Geometry check sheet. Reference: the model listing, model coordinates, mm. Face numbers are marked on the shaded views. A direction names the side the tool comes from. Give positions to 0.01 mm unless a question says otherwise; leave off trailing zeros. Write each loop counter-clockwise with the first axis right and the second up, starting at its lowest first coordinate (ties: lowest second). Pieces come first, ordered by that corner, then holes. Notation, with made-up numbers: (12, -4.5) -> (16, -4.5) arc R19 ccw to (16, 26.5) -> close; hole circle Ø7 at (-30, 23.5). An arc over 180 degrees is marked (long way). Use a Markdown table: item, result. Add a question column.
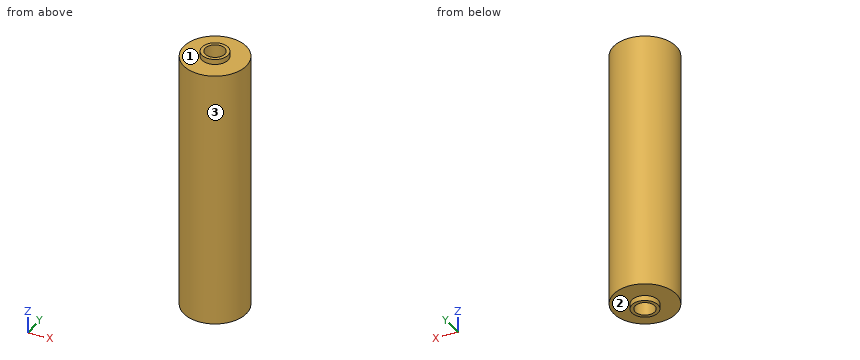
from build123d import *

# Parameters (mm, degrees)
SKETCH_1_R          = 120
EXTRUDE_1_DEPTH     = 1000
SKETCH_2_R          = 37.5
CUT_EXTRUDE_1_DEPTH = 1000
EXTRUDE_START       = 20
SKETCH_3_R          = 50
SKETCH_3_R_2        = 37.5
EXTRUDE_2_DEPTH     = 20


with BuildPart() as part:
    # 草图1 → 凸台-拉伸1 (new body)
    with BuildSketch(Plane.XY):
        Circle(SKETCH_1_R)
    extrude(amount=EXTRUDE_1_DEPTH)

    # 草图2 → 切除-拉伸1 (cut)
    with BuildSketch(Plane.XY.offset(1000)):
        Circle(SKETCH_2_R)
    extrude(amount=-CUT_EXTRUDE_1_DEPTH, mode=Mode.SUBTRACT)

    # 草图3 → 凸台-拉伸2 (add)
    with BuildSketch(Plane.XY.offset(1000).offset(EXTRUDE_START)):
        Circle(SKETCH_3_R)
        Circle(SKETCH_3_R_2, mode=Mode.SUBTRACT)
    extrude_2 = extrude(amount=-EXTRUDE_2_DEPTH)

    # 镜向1: 凸台-拉伸2 across plane
    add(extrude_2.mirror(Plane.XY.offset(500)))


solid = part.part
1) Sectioned sample at D-D, the plane y = 71. Enter the section's corners in (x, z), and give its area (3 significant figures).
2) Sectioned sample at C-C, the plane z = 709. Enter the section's corners in (x, y).
3) Tool access check on the marked faces 1, 2 and 3. Record the directions out of +Z, -Z, +X, -X, +Y, -Y that give a thin tool (end or side, any length) a straight path to the whole face; none if there is none.
4) Sectioned sample at A-A, the plane x = 0. Enter the section's corners in (y, z), and give its area (3 significant figures).
5) Gauge pin test, flat ends, axial feed: P1, Ø8, axis at x = 80.5, z = 148, coming from the +Y side; P2, Ø1, axis at x = 65.5, z = 460, coming from the -Y side; P3, Ø12, axis at x = -15.5, z = 143.5, coming from the -Y side. Record the tip position at first contact, or that the pin passes through.
6) Material ranges on probe 1 along Y at (x, z) = (0, 402.5); probe 2 along Y at (x, z) = (2, 289); probe 3 along Z at (x, y) = (44.5, 95.5), recorded low to high. Write a range as [from, to].
Check values:
| question | item | result |
|---|---|---|
| 1 | outline | (-96.74, 0) -> (96.74, 0) -> (96.74, 1000) -> (-96.74, 1000) -> close |
| 1 | area | 193,000 mm² |
| 2 | outline | circle Ø240 at (0, 0); hole circle Ø75 at (0, 0) |
| 3 | face 1 | +Z |
| 3 | face 2 | -Z |
| 3 | face 3 | +Z, -Z |
| 4 | outline | (-120, 0) -> (-50, 0) -> (-50, -20) -> (-37.5, -20) -> (-37.5, 1020) -> (-50, 1020) -> (-50, 1000) -> (-120, 1000) -> close; (37.5, -20) -> (50, -20) -> (50, 0) -> (120, 0) -> (120, 1000) -> (50, 1000) -> (50, 1020) -> (37.5, 1020) -> close |
| 4 | area | 166,000 mm² |
| 5 | P1 | y = 92.45 |
| 5 | P2 | y = -100.87 |
| 5 | P3 | y = -119.62 |
| 6 | probe 1 | [-120, -37.5], [37.5, 120] |
| 6 | probe 2 | [-119.98, -37.45], [37.45, 119.98] |
| 6 | probe 3 | [0, 1000] |
